```python
from build123d import *

# Parameters (mm, degrees)
SKETCH1_R           = 3
SKETCH1_R_2         = 1.5
BOSS_EXTRUDE1_DEPTH = 5


with BuildPart() as part:
    # Sketch1 → Boss-Extrude1 (new body)
    with BuildSketch(Plane.XY):
        Polygon((-10, -10), (-10, 10), (-5, 10), (5, 10), (10, 10), (10, -10), (10, -13), (3.5, -13), (3.5, -9.2), (-3.5, -9.2), (-3.5, -13), (-10, -13), align=None)
        Circle(SKETCH1_R, mode=Mode.SUBTRACT)
        with Locations((-7, 7)):
            Circle(SKETCH1_R_2, mode=Mode.SUBTRACT)
        with Locations((7, 7)):
            Circle(SKETCH1_R_2, mode=Mode.SUBTRACT)
        with Locations((7, -7)):
            Circle(SKETCH1_R_2, mode=Mode.SUBTRACT)
        with Locations((-7, -7)):
            Circle(SKETCH1_R_2, mode=Mode.SUBTRACT)
    extrude(amount=BOSS_EXTRUDE1_DEPTH)


solid = part.part
```
The listing builds one solid part. Answer for the finished solid, in the listing's coordinates (mm). A direction names the side the tool comes from. Coordinates: 2 decimals unless noted, no trailing zeros. Write each loop counter-clockwise with the first axis right and the second up, starting at its lowest first coordinate (ties: lowest second). Pieces come first, ordered by that corner, then holes. Notation, with made-up numbers: (7.25, -33.5) -> (62.25, -33.5) arc R11 ccw to (62.25, -26.5) -> close; hole circle Ø1 at (23.5, -8.75). An arc over 180 degrees is marked (long way). Write each question's results on one line, items separated by ' | '. Start each with the question number.
1) A tool of negligible diameter and unlimited length cuts with its end or side. For faces 1 (the cylindrical face through (-3, 0, 2)), 2 (the flat face through (-3.5, -11, 2)), from which of +Z, -Z, +X, -X, +Y, -Y can it reach the whole face along a straight path? Write none if from no direction.
2) A cutting plane is placed at D-D (y = 0). Determine the outline of the cut face in (x, z), then the cut area to 3 significant figures.
3) A cutting plane is placed at B-B (y = 7). Determine the outline of the cut face in (x, z).
4) A flat-ended cylindrical pin translates along its axis: pin 1 Ø2.5 at (x, z) = (1.5, 1.5) entering from -Y. Find the tip coordinate at first contact, or state that the pin passes through.
5) For a pull along X with two mould halves and no side action, classify faces 3 (the flat face through (0, -4, 5)), 4 (the flat face through (3.5, -11, 2)), 5 (the flat face through (-10, -1, 2)) as +X half, -X half, draft (parallel to the pull), parting line (faces both ways), or undercut.
6) A cutting plane is placed at C-C (z = 1.2). Determine the outline of the cut face in (x, y).
7) Straight lines are drawn through the part: probe 1 along Y at (x, z) = (7, 3); probe 2 along X at (y, z) = (-11.5, 1.3); probe 3 along Y at (x, z) = (0, 2). For each, find the intervals that lie inside material, in ascending order.
8) A cutting plane is placed at A-A (x = -7). Determine the outline of the cut face in (y, z), then the cut area to 3 significant figures.
Values follow:
1) face 1: +Z, -Z | face 2: +Z, -Z, -Y
2) outline: (-10, 0) -> (-3, 0) -> (-3, 5) -> (-10, 5) -> close; (3, 0) -> (10, 0) -> (10, 5) -> (3, 5) -> close | area: 70.0 mm²
3) outline: (-10, 0) -> (-8.5, 0) -> (-8.5, 5) -> (-10, 5) -> close; (-5.5, 0) -> (5.5, 0) -> (5.5, 5) -> (-5.5, 5) -> close; (8.5, 0) -> (10, 0) -> (10, 5) -> (8.5, 5) -> close
4) pin 1: y = -9.2
5) face 3: draft | face 4: undercut | face 5: -X half
6) outline: (-10, -13) -> (-3.5, -13) -> (-3.5, -9.2) -> (3.5, -9.2) -> (3.5, -13) -> (10, -13) -> (10, 10) -> (-10, 10) -> close; hole circle Ø3 at (-7, -7); hole circle Ø3 at (-7, 7); hole circle Ø6 at (0, 0); hole circle Ø3 at (7, -7); hole circle Ø3 at (7, 7)
7) probe 1: -13 to -8.5, -5.5 to 5.5, 8.5 to 10 | probe 2: -10 to -3.5, 3.5 to 10 | probe 3: -9.2 to -3, 3 to 10
8) outline: (-13, 0) -> (-8.5, 0) -> (-8.5, 5) -> (-13, 5) -> close; (-5.5, 0) -> (5.5, 0) -> (5.5, 5) -> (-5.5, 5) -> close; (8.5, 0) -> (10, 0) -> (10, 5) -> (8.5, 5) -> close | area: 85.0 mm²
